```python
from build123d import *
from OCP.BRepFilletAPI import BRepFilletAPI_MakeChamfer

# Parameters (mm, degrees)
SKETCH1_R           = 19
SKETCH1_R_2         = 12.5
BOSS_EXTRUDE1_DEPTH = 6
SKETCH2_W           = 6
SKETCH2_H           = 4
CUT_EXTRUDE1_DEPTH  = 6
CIRPATTERN1_COUNT   = 4
CHAMFER1_SIZE       = 0.5
CHAMFER2_SIZE       = 2
CHAMFER2_SIZE2      = 1.154700538


with BuildPart() as part:
    # Sketch1 → Boss-Extrude1 (new body)
    with BuildSketch(Plane.XY):
        Circle(SKETCH1_R)
        Circle(SKETCH1_R_2, mode=Mode.SUBTRACT)
    extrude(amount=BOSS_EXTRUDE1_DEPTH)

    # Sketch2 → Cut-Extrude1 (cut)
    with BuildSketch(Plane(origin=(14, 0, 0), x_dir=(0, 0, -1), z_dir=(1, 0, 0))):
        with Locations((-3, 0)):
            Rectangle(SKETCH2_W, SKETCH2_H)
    cut_extrude1 = extrude(amount=CUT_EXTRUDE1_DEPTH, mode=Mode.SUBTRACT)

    # CirPattern1: Cut-Extrude1 ×4 about axis
    cirpattern1_axis = Axis((0, 0, 0), (0, 0, 1))
    for i in range(1, CIRPATTERN1_COUNT):
        add(cut_extrude1.rotate(cirpattern1_axis, i * 360 / CIRPATTERN1_COUNT), mode=Mode.SUBTRACT)

    # Chamfer1
    chamfer1_edges = [part.edges().sort_by_distance(p)[0] for p in [
        (-12.5, 0, 0),
        (-12.5, 0, 6),
    ]]
    chamfer(chamfer1_edges, length=CHAMFER1_SIZE)

    # Chamfer2: one chamfer whose edges measure the first distance from different faces: ONE call of the kernel's chamfer builder (chamfer() names one face for all edges)
    chamfer2_edges_1 = [part.edges().sort_by_distance(p)[0] for p in [
        (13.435028843, -13.435028843, 6),
    ]]
    chamfer2_side_1 = [part.faces().sort_by_distance(p)[0] for p in [
        (13.435028843, -13.435028843, 3),
    ]]
    chamfer2_edges_2 = [part.edges().sort_by_distance(p)[0] for p in [
        (13.435028843, 13.435028843, 6),
    ]]
    chamfer2_side_2 = [part.faces().sort_by_distance(p)[0] for p in [
        (13.435028843, 13.435028843, 3),
    ]]
    chamfer2_edges_3 = [part.edges().sort_by_distance(p)[0] for p in [
        (-13.435028843, -13.435028843, 6),
    ]]
    chamfer2_side_3 = [part.faces().sort_by_distance(p)[0] for p in [
        (-13.435028843, -13.435028843, 3),
    ]]
    chamfer2_edges_4 = [part.edges().sort_by_distance(p)[0] for p in [
        (-13.435028843, 13.435028843, 6),
    ]]
    chamfer2_side_4 = [part.faces().sort_by_distance(p)[0] for p in [
        (-13.435028843, 13.435028843, 3),
    ]]
    chamfer2 = BRepFilletAPI_MakeChamfer(part.part.solid().wrapped)
    for e in chamfer2_edges_1:
        chamfer2.Add(CHAMFER2_SIZE, CHAMFER2_SIZE2, e.wrapped, chamfer2_side_1[0].wrapped)  # the first distance lies on this face
    for e in chamfer2_edges_2:
        chamfer2.Add(CHAMFER2_SIZE, CHAMFER2_SIZE2, e.wrapped, chamfer2_side_2[0].wrapped)  # the first distance lies on this face
    for e in chamfer2_edges_3:
        chamfer2.Add(CHAMFER2_SIZE, CHAMFER2_SIZE2, e.wrapped, chamfer2_side_3[0].wrapped)  # the first distance lies on this face
    for e in chamfer2_edges_4:
        chamfer2.Add(CHAMFER2_SIZE, CHAMFER2_SIZE2, e.wrapped, chamfer2_side_4[0].wrapped)  # the first distance lies on this face
    add(Compound.cast(chamfer2.Shape()), mode=Mode.REPLACE)


solid = part.part
```
Geometry check sheet. Reference: the model listing, model coordinates, mm. A direction names the side the tool comes from. Round coordinates to 2 decimals unless told otherwise and drop trailing zeros. Write each loop counter-clockwise with the first axis right and the second up, starting at its lowest first coordinate (ties: lowest second). Pieces come first, ordered by that corner, then holes. Notation, with made-up numbers: (56.25, -14.5) - (112.25, -14.5) arc R12 cw to (112.25, 4.5) - close; hole circle Ø10 at (64.25, 38). An arc over 180 degrees is marked (long way). Write each question's results on one line, items separated by ' | '.
(1) Thickness scan on probe 1 along Y at (x, z) = (0, 3.1); probe 2 along Y at (x, z) = (6, 1); probe 3 along X at (y, z) = (5, 0.75). Record the ranges inside material, lowest first. Write a range as from..to.
Computed:
probe 1: y = -14..-12.5, 12.5..14 | probe 2: y = -18.03..-10.97, 10.97..18.03 | probe 3: x = -18.33..-11.46, 11.46..18.33
(2) Depth check by flat-ended pin: pin 1 Ø1.5 at (y, z) = (-9, 2.5) entering from +X; pin 2 Ø1.5 at (x, y) = (-12.5, -0.5) entering from -Z; pin 3 Ø1.5 at (x, z) = (-16.5, 3.5) entering from -Y; pin 4 Ø3 at (x, z) = (11.5, 1) entering from +Y. Enter the tip coordinate at first touch or a pass-through.
Computed:
pin 1: stops at x = 17.12 | pin 2: stops at z = 0 | pin 3: stops at y = -10.63 | pin 4: stops at y = 16.16
(3) Set-up check for faces 1 (the face through (14, 0, 3)), 2 (the face through (13.31, -13.56, 1.97)), 3 (the face through (-2, -16, 3)), 4 (the face through (2, 16, 3)): record each of +Z, -Z, +X, -X, +Y, -Y from which the full face is reachable in a straight line by a thin tool's end or side.
Computed:
face 1: +Z, -Z, +X | face 2: +Z, -Z, +X, -Y | face 3: +Z, -Z, -Y | face 4: +Z, -Z, +Y
(4) Sectioned sample at A-A, the plane x = 0. Enter the section's corners in (y, z), plus the area to 3 significant figures.
Computed:
outline: (-14, 0) - (-13, 0) - (-12.5, 0.5) - (-12.5, 5.5) - (-13, 6) - (-14, 6) - close; (12.5, 0.5) - (13, 0) - (14, 0) - (14, 6) - (13, 6) - (12.5, 5.5) - close | area: 17.5 mm^2
(5) Sectioned sample at C-C, the plane z = 1.25. Enter the section's corners in (x, y), plus the area to 3 significant figures.
Computed:
outline: (-18.89, -2) arc R19 ccw to (-2, -18.89) - (-2, -14) - (2, -14) - (2, -18.89) arc R19 ccw to (18.89, -2) - (14, -2) - (14, 2) - (18.89, 2) arc R19 ccw to (2, 18.89) - (2, 14) - (-2, 14) - (-2, 18.89) arc R19 ccw to (-18.89, 2) - (-14, 2) - (-14, -2) - close; hole circle Ø25 at (0, 0) | area: 564 mm^2
(6) Draft check along X on faces 5 (the face through (12.63, -12.87, 5.68)), 6 (the face through (-13, -4, 0)), 7 (the face through (0, -14, 3)). Enter one of: pulls with the +X half, pulls with the -X half, needs draft (parallel to the pull), parting line crosses it, or undercut.
Computed:
face 5: pulls with the +X half | face 6: needs draft | face 7: undercut
